Verification items for the finished model (mm, model axes). A direction names the side the tool comes from. Give positions to 0.01 mm unless a question says otherwise; leave off trailing zeros. Loops run counter-clockwise (first coordinate to the right, second up) from the corner with the lowest first, then second, coordinate; pieces in that order, holes last. Notation, with made-up numbers: M 1.25,-36 L 7.25,-36 A12 cw 7.25,-28 Z; hole C 26.5,45.25 d9. An arc over 180 degrees is marked long. Use a Markdown table: item, result.
from build123d import *

# Parameters (mm, degrees)
SKETCH_1_W                   = 23
SKETCH_1_H                   = 20
EXTRUDE_1_DEPTH              = 11
HOLE_WIZARD_M6_1_D           = 6.6
HOLE_WIZARD_M6_1_CBORE_D     = 11
HOLE_WIZARD_M6_1_CBORE_DEPTH = 6.4
CHAMFER_1_SIZE               = 1


with BuildPart() as part:
    # 草图1 → 凸台-拉伸1 (new, symmetric)
    with BuildSketch(Plane(origin=(0, 0, 0), x_dir=(1, 0, 0), z_dir=(0, 1, 0))):
        Rectangle(SKETCH_1_W, SKETCH_1_H)
    extrude(amount=EXTRUDE_1_DEPTH, both=True)

    # M6 六角凹头螺钉的柱形沉头孔1 (through all)
    with Locations(Plane(origin=(0, 11, 0), x_dir=(1, 0, 0), z_dir=(0, 1, 0))):
        with Locations((0, 0)):
            CounterBoreHole(HOLE_WIZARD_M6_1_D / 2, HOLE_WIZARD_M6_1_CBORE_D / 2, HOLE_WIZARD_M6_1_CBORE_DEPTH)

    # 倒角1
    chamfer_1_edges = [part.edges().sort_by_distance(p)[0] for p in [
        (-11.5, 0, -10),
        (11.5, 0, -10),
        (11.5, 0, 10),
        (-11.5, 0, 10),
    ]]
    chamfer(chamfer_1_edges, length=CHAMFER_1_SIZE)


solid = part.part
(1) Cross-section at A-A on x = 0. Record the cut outline in (y, z).
Results below:
| item | result |
|---|---|
| outline | M -11,-10 L 11,-10 L 11,-5.5 L 4.6,-5.5 L 4.6,-3.3 L -11,-3.3 Z; M -11,3.3 L 4.6,3.3 L 4.6,5.5 L 11,5.5 L 11,10 L -11,10 Z |
(2) Cross-section at C-C on y = 5. Record the cut outline in (x, z).
Results below:
| item | result |
|---|---|
| outline | M -11.5,-9 L -10.5,-10 L 10.5,-10 L 11.5,-9 L 11.5,9 L 10.5,10 L -10.5,10 L -11.5,9 Z; hole C 0,0 d11 |
(3) Gauge pin test, flat end, axial feed: P1, Ø9, axis at x = 0, z = 0, coming from the +Y side. Record the tip position at first contact, or that the pin passes through.
Results below:
| item | result |
|---|---|
| P1 | y = 4.6 |
(4) Draft check along Z on faces 1 (the cylindrical face through (2.43, -3.31, -2.23)), 2 (the flat face through (-11, -0.2, 9.5)), 3 (the flat face through (-11, 0.2, -9.5)). Enter one of: +Z half, -Z half, draft (parallel to the pull), parting line (faces both ways), or undercut.
Results below:
| item | result |
|---|---|
| face 1 | undercut |
| face 2 | +Z half |
| face 3 | -Z half |
(5) Set-up check for faces 4 (the cylindrical face through (-1.19, 7.84, 5.37)), 5 (the flat face through (0, 0, -10)): record each of +Z, -Z, +X, -X, +Y, -Y from which the full face is reachable in a straight line by a thin tool's end or side.
Results below:
| item | result |
|---|---|
| face 4 | +Y |
| face 5 | -Z, +X, -X, +Y, -Y |
(6) Material ranges on line 1 (Z direction, x = 0, y = 6); line 2 (Z direction, x = 0, y = -3.5); line 3 (Y direction, x = -2.75, z = -2.5), recorded low to high.
Results below:
| item | result |
|---|---|
| line 1 | -10 to -5.5, 5.5 to 10 |
| line 2 | -10 to -3.3, 3.3 to 10 |
| line 3 | -11 to 4.6 |
(7) Cross-section at D-D on y = -6. Record the cut outline in (x, z), then the cut area to 3 significant figures.
Results below:
| item | result |
|---|---|
| outline | M -11.5,-9 L -10.5,-10 L 10.5,-10 L 11.5,-9 L 11.5,9 L 10.5,10 L -10.5,10 L -11.5,9 Z; hole C 0,0 d6.6 |
| area | 424 mm^2 |
(8) Cross-section at B-B on z = 0. Record the cut outline in (x, y), then the cut area to 3 significant figures.
Results below:
| item | result |
|---|---|
| outline | M -11.5,-11 L -3.3,-11 L -3.3,4.6 L -5.5,4.6 L -5.5,11 L -11.5,11 Z; M 3.3,-11 L 11.5,-11 L 11.5,11 L 5.5,11 L 5.5,4.6 L 3.3,4.6 Z |
| area | 333 mm^2 |
